```python
from build123d import *

# Parameters (mm, degrees)
BASE_PLATE_SKETCH_W             = 150
BASE_PLATE_SKETCH_H             = 80
BASE_PLATE_DEPTH                = 15
PROFILE_TRIM_CUT_DEPTH          = 35
COUNTERBORE_SKETCH_R            = 12.5
COUNTERBORE_SKETCH_R_2          = 6
COUNTERBORE_25X5_DEPTH          = 5
THROUGH_HOLE_SKETCH_R           = 6
THROUGH_HOLE_CUT_DEPTH          = 25
ARC_SLOT_8_R50_30DEG_DEPTH      = 86.586213843
ARC_SLOT_8_R50_30DEG_DEPTH_BACK = 86.586213843
UPRIGHT_FLANGE_SKETCH_R         = 7.5
UPRIGHT_FLANGE_DEPTH            = 15


with BuildPart() as part:
    # Base Plate Sketch → Base Plate (new body)
    with BuildSketch(Plane(origin=(0, 0, 0), x_dir=(1, 0, 0), z_dir=(0, 1, 0))):
        Rectangle(BASE_PLATE_SKETCH_W, BASE_PLATE_SKETCH_H)
    extrude(amount=BASE_PLATE_DEPTH)

    # Profile Trim Sketch → Profile Trim Cut (cut)
    with BuildSketch(Plane(origin=(0, 15, 0), x_dir=(1, 0, 0), z_dir=(0, 1, 0))):
        with BuildLine():
            Line((75, 0), (75, 40))
            Line((75, 40), (63.442887702, 40))
            ThreePointArc((63.442887702, 40), (72.052815967, 20.818062138), (75, 0))
        make_face()
        with BuildLine():
            Line((75, -40), (75, 0))
            ThreePointArc((75, 0), (72.052815967, -20.818062138), (63.442887702, -40))
            Line((63.442887702, -40), (75, -40))
        make_face()
    extrude(amount=-PROFILE_TRIM_CUT_DEPTH, mode=Mode.SUBTRACT)

    # Counterbore Sketch → Counterbore Ø25x5 (cut)
    with BuildSketch(Plane(origin=(0, 15, 0), x_dir=(1, 0, 0), z_dir=(0, 1, 0))):
        with Locations(Location((0, 0, 0), (0, 0, 270))):
            Circle(COUNTERBORE_SKETCH_R)
        with Locations(Location((0, 0, 0), (0, 0, 270))):
            Circle(COUNTERBORE_SKETCH_R_2, mode=Mode.SUBTRACT)
    extrude(amount=-COUNTERBORE_25X5_DEPTH, mode=Mode.SUBTRACT)

    # Through Hole Sketch → Through Hole Cut (cut)
    with BuildSketch(Plane(origin=(0, 15, 0), x_dir=(1, 0, 0), z_dir=(0, 1, 0))):
        with Locations(Location((0, 0, 0), (0, 0, 270))):
            Circle(THROUGH_HOLE_SKETCH_R)
    extrude(amount=-THROUGH_HOLE_CUT_DEPTH, mode=Mode.SUBTRACT)

    # Arc Slot Sketch → Arc Slot 8 R50 30deg (cut, two sides: drawn at the far end of the back side and taken through both)
    with BuildSketch(Plane(origin=(0, 10, 0), x_dir=(1, 0, 0), z_dir=(0, 1, 0)).offset(-ARC_SLOT_8_R50_30DEG_DEPTH_BACK)):
        with BuildLine():
            ThreePointArc((50.229473419, -29), (58, 0), (50.229473419, 29))
            ThreePointArc((50.229473419, 29), (39.301270189, 31.92820323), (36.373066959, 21))
            ThreePointArc((36.373066959, 21), (42, 0), (36.373066959, -21))
            ThreePointArc((36.373066959, -21), (39.301270189, -31.92820323), (50.229473419, -29))
        make_face()
    extrude(amount=ARC_SLOT_8_R50_30DEG_DEPTH + ARC_SLOT_8_R50_30DEG_DEPTH_BACK, mode=Mode.SUBTRACT)

    # Upright Flange Sketch → Upright Flange (add)
    with BuildSketch(Plane.ZY.offset(75)):
        with BuildLine():
            Line((-40, 15), (-40, 55))
            ThreePointArc((-40, 55), (-34.142135624, 69.142135624), (-20, 75))
            Line((-20, 75), (20, 75))
            ThreePointArc((20, 75), (34.142135624, 69.142135624), (40, 55))
            Line((40, 55), (40, 15))
            Line((40, 15), (-40, 15))
        make_face()
        with Locations((-20, 55)):
            Circle(UPRIGHT_FLANGE_SKETCH_R, mode=Mode.SUBTRACT)
        with Locations((20, 55)):
            Circle(UPRIGHT_FLANGE_SKETCH_R, mode=Mode.SUBTRACT)
    extrude(amount=-UPRIGHT_FLANGE_DEPTH)


solid = part.part
```
Geometry check sheet. Reference: the model listing, model coordinates, mm. A direction names the side the tool comes from. Round coordinates to 2 decimals unless told otherwise and drop trailing zeros. Order: outer loops, then holes, each group sorted by start corner. A loop starts at its lowest first (then second) coordinate and runs counter-clockwise, first axis right, second up. Notation, with made-up numbers: (11, -6.75) -> (42, -6.75) arc R23 cw to (42, 1.25) -> close; hole circle Ø8 at (63, 30.5). An arc over 180 degrees is marked (long way). Return JSON: item names as keys, results as strings. Group by question number.
Q1. Gauge pin test, flat ends, axial feed: pin 1 (8 mm diameter, centred on y = 45.5, z = 7, fed in from +X); pin 2 (6 mm diameter, centred on x = 27, z = 9, fed in from +Y); pin 3 (12 mm diameter, centred on y = 55, z = -20, fed in from +X); pin 4 (7.5 mm diameter, centred on x = 6, z = 4.5, fed in from +Y). Record the tip position at first contact, or that the pin passes through.
Q2. Tool access check on faces 5 (the cylindrical face through (58, 7, 0)), 6 (the flat face through (3, 10, 5.4)), 7 (the flat face through (-8.44, 15, -9.45)). Record the directions out of +Z, -Z, +X, -X, +Y, -Y that give a thin tool (end or side, any length) a straight path to the whole face; none if there is none.
Q3. Section check A-A, the plane x = 0. Record the boundary of the cut face in (y, z), plus the area to 3 significant figures.
Q4. Section check C-C, the plane y = 30.5. Record the boundary of the cut face in (x, z).
Q5. Section check B-B, the plane z = -7.5. Record the boundary of the cut face in (x, y).
Q6. Section check D-D, the plane x = 54.5. Record the boundary of the cut face in (y, z), plus the area to 3 significant figures.
Q7. Release check for a two-part mould opening along Z. For faces 1 (the cylindrical face through (-67.605, 69.297, 33.986)), 2 (the cylindrical face through (3.755, 12.535, 11.923)), 3 (the flat face through (-68, 75, 0)), 4 (the cylindrical face through (42, 7, 0)) record: released by +Z, released by -Z, zero draft, split by the parting line, or undercut.
Q8. Material ranges on probe 1 along Y at (x, z) = (-64.25, 20); probe 2 along X at (y, z) = (28, -20); probe 3 along X at (y, z) = (14, -30), recorded low to high. Write a range as from..to.
Numbers:
{
 "1": {"pin 1": "x = -60", "pin 2": "y = 15", "pin 3": "through", "pin 4": "y = 10"},
 "2": {"face 5": "+Y, -Y", "face 6": "+Y", "face 7": "+Z, -Z, +X, +Y"},
 "3": {"outline": "(0, -40) -> (15, -40) -> (15, -12.5) -> (10, -12.5) -> (10, -6) -> (0, -6) -> close; (0, 6) -> (10, 6) -> (10, 12.5) -> (15, 12.5) -> (15, 40) -> (0, 40) -> close", "area": "955 mm^2"},
 "4": {"outline": "(-75, -40) -> (-60, -40) -> (-60, 40) -> (-75, 40) -> close"},
 "5": {"outline": "(-75, 0) -> (41.32, 0) -> (41.32, 15) -> (10, 15) -> (10, 10) -> (-10, 10) -> (-10, 15) -> (-60, 15) -> (-60, 75) -> (-75, 75) -> close; (57.51, 0) -> (74.62, 0) -> (74.62, 15) -> (57.51, 15) -> close"},
 "6": {"outline": "(0, -40) -> (15, -40) -> (15, -19.84) -> (0, -19.84) -> close; (0, 19.84) -> (15, 19.84) -> (15, 40) -> (0, 40) -> close", "area": "605 mm^2"},
 "7": {"face 1": "released by +Z", "face 2": "undercut", "face 3": "zero draft", "face 4": "undercut"},
 "8": {"probe 1": "0..47.5, 62.5..75", "probe 2": "-75..-60", "probe 3": "-75..37.06, 49.55..68.74"}
}
